Input: part model. Units: mm. Frame: model coordinates. A direction names the side the tool comes from. Round coordinates to 2 decimals unless told otherwise and drop trailing zeros. Loops run counter-clockwise (first coordinate to the right, second up) from the corner with the lowest first, then second, coordinate; pieces in that order, holes last.
1) Access query for faces 4 (the face through (2.86, -0.9, -14.47)), 5 (the face through (-1.267, -2.155, 5.231)), 6 (the face through (2, 2, 6)). Directions: +Z, -Z, +X, -X, +Y, -Y. A direction counts if a zero-diameter tool reaches every point of the face in a straight line with its end or side. Return the directions, or none.
2) Draft query along Y for faces 1 (the face through (-0.74, 1.32, 3.87)), 2 (the face through (0, 0, -30)), 3 (the face through (-1.08, -4.88, 2.58)). Return one class per face: pulls with the +Y half, pulls with the -Y half, needs draft (parallel to the pull), parting line crosses it, or undercut.
3) First-contact query: pin 1 (4 mm diameter, centred on x = 0, z = -7, fed in from -Y); pin 2 (3 mm diameter, centred on y = 0, z = -14.5, fed in from -X); pin 3 (6 mm diameter, centred on y = 4, z = -22, fed in from -X). Flat tips, straight axial feed; report the tip coordinate or a pass-through.
4) Section A-A, the plane z = -1.5. Return loops of the section in (x, y), and give its area (3 significant figures).
5) Ray query, line 1 along Z through (x, y) = (3.25, 0.5); line 2 along Y through (x, z) = (0, -16.5); line 3 along Y through (x, z) = (-4.5, 4). Return the intervals inside material, ascending.
from build123d import *
from OCP.BRepFilletAPI import BRepFilletAPI_MakeChamfer

# Parameters (mm, degrees)
SKETCH1_R           = 5
BOSS_EXTRUDE1_DEPTH = 6
CUT_EXTRUDE1_DEPTH  = 3
SKETCH3_R           = 3
BOSS_EXTRUDE2_DEPTH = 30
CHAMFER1_SIZE       = 0.75
FILLET1_R           = 0.769230769
CHAMFER2_SIZE       = 1.44092219
CHAMFER2_SIZE2      = 2.495750443
FILLET2_R           = 0.1


with BuildPart() as part:
    # Sketch1 → Boss-Extrude1 (new body)
    with BuildSketch(Plane.XY):
        Circle(SKETCH1_R)
    extrude(amount=BOSS_EXTRUDE1_DEPTH)

    # Sketch2 → Cut-Extrude1 (cut)
    with BuildSketch(Plane.XY.offset(6)):
        Polygon((2.5, 1.443375673), (0, 2.886751346), (-2.5, 1.443375673), (-2.5, -1.443375673), (0, -2.886751346), (2.5, -1.443375673), align=None)
    extrude(amount=-CUT_EXTRUDE1_DEPTH, mode=Mode.SUBTRACT)

    # Sketch3 → Boss-Extrude2 (add)
    with BuildSketch(Plane(origin=(0, 0, 0), x_dir=(-1, 0, 0), z_dir=(0, 0, -1))):
        with Locations(Location((0, 0, 0), (0, 0, 180))):
            Circle(SKETCH3_R)
    extrude(amount=BOSS_EXTRUDE2_DEPTH)

    # Chamfer1
    chamfer1_edges = [part.edges().sort_by_distance(p)[0] for p in [
        (-3, 0, -30),
    ]]
    chamfer(chamfer1_edges, length=CHAMFER1_SIZE)

    # Fillet1
    fillet1_edges = [part.edges().sort_by_distance(p)[0] for p in [
        (-5, 0, 6),
    ]]
    fillet(fillet1_edges, radius=FILLET1_R)

    # Chamfer2: one chamfer whose edges measure the first distance from different faces: ONE call of the kernel's chamfer builder (chamfer() names one face for all edges)
    chamfer2_edges_1 = [part.edges().sort_by_distance(p)[0] for p in [
        (-1.25, 2.165063509, 3),
    ]]
    chamfer2_side_1 = [part.faces().sort_by_distance(p)[0] for p in [
        (-1.25, 2.165063509, 4.5),
    ]]
    chamfer2_edges_2 = [part.edges().sort_by_distance(p)[0] for p in [
        (1.25, 2.165063509, 3),
    ]]
    chamfer2_side_2 = [part.faces().sort_by_distance(p)[0] for p in [
        (1.25, 2.165063509, 4.5),
    ]]
    chamfer2_edges_3 = [part.edges().sort_by_distance(p)[0] for p in [
        (2.5, 0, 3),
    ]]
    chamfer2_side_3 = [part.faces().sort_by_distance(p)[0] for p in [
        (2.5, 0, 4.5),
    ]]
    chamfer2_edges_4 = [part.edges().sort_by_distance(p)[0] for p in [
        (1.25, -2.165063509, 3),
    ]]
    chamfer2_side_4 = [part.faces().sort_by_distance(p)[0] for p in [
        (1.25, -2.165063509, 4.5),
    ]]
    chamfer2_edges_5 = [part.edges().sort_by_distance(p)[0] for p in [
        (-1.25, -2.165063509, 3),
    ]]
    chamfer2_side_5 = [part.faces().sort_by_distance(p)[0] for p in [
        (-1.25, -2.165063509, 4.5),
    ]]
    chamfer2_edges_6 = [part.edges().sort_by_distance(p)[0] for p in [
        (-2.5, 0, 3),
    ]]
    chamfer2_side_6 = [part.faces().sort_by_distance(p)[0] for p in [
        (-2.5, 0, 4.5),
    ]]
    chamfer2 = BRepFilletAPI_MakeChamfer(part.part.solid().wrapped)
    for e in chamfer2_edges_1:
        chamfer2.Add(CHAMFER2_SIZE, CHAMFER2_SIZE2, e.wrapped, chamfer2_side_1[0].wrapped)  # the first distance lies on this face
    for e in chamfer2_edges_2:
        chamfer2.Add(CHAMFER2_SIZE, CHAMFER2_SIZE2, e.wrapped, chamfer2_side_2[0].wrapped)  # the first distance lies on this face
    for e in chamfer2_edges_3:
        chamfer2.Add(CHAMFER2_SIZE, CHAMFER2_SIZE2, e.wrapped, chamfer2_side_3[0].wrapped)  # the first distance lies on this face
    for e in chamfer2_edges_4:
        chamfer2.Add(CHAMFER2_SIZE, CHAMFER2_SIZE2, e.wrapped, chamfer2_side_4[0].wrapped)  # the first distance lies on this face
    for e in chamfer2_edges_5:
        chamfer2.Add(CHAMFER2_SIZE, CHAMFER2_SIZE2, e.wrapped, chamfer2_side_5[0].wrapped)  # the first distance lies on this face
    for e in chamfer2_edges_6:
        chamfer2.Add(CHAMFER2_SIZE, CHAMFER2_SIZE2, e.wrapped, chamfer2_side_6[0].wrapped)  # the first distance lies on this face
    add(Compound.cast(chamfer2.Shape()), mode=Mode.REPLACE)

    # Fillet2
    fillet2_edges = [part.edges().sort_by_distance(p)[0] for p in [
        (-3, 0, 0),
    ]]
    fillet(fillet2_edges, radius=FILLET2_R)


solid = part.part
Final values:
1. face 4: -Z
1. face 5: +Z
1. face 6: +Z, +X, -X, +Y, -Y
2. face 1: undercut
2. face 2: needs draft
2. face 3: parting line crosses it
3. pin 1: stops at y = -3
3. pin 2: stops at x = -3
3. pin 3: stops at x = -2.83
4. outline: circle Ø6 at (0, 0)
4. area: 28.3 mm2
5. line 1: z = 0 to 6
5. line 2: y = -3 to 3
5. line 3: y = -2.18 to 2.18
